Part model, mm, in its own coordinate system. Round coordinates to 2 decimals unless told otherwise and drop trailing zeros. Loops run counter-clockwise (first coordinate to the right, second up) from the corner with the lowest first, then second, coordinate; pieces in that order, holes last. Notation, with made-up numbers: (-17.75, -10) - (35.25, -10) arc R22 ccw to (35.25, 20) - close; hole circle Ø1 at (58.25, 21). An arc over 180 degrees is marked (long way). Write each question's results on one line, items separated by ' | '. Start each with the question number.
(1) Flat gauge pins, fed straight in: P1, Ø6, axis at y = -9, z = -19, coming from the +X side; P2, Ø8, axis at x = 182.5, y = 3, coming from the -Z side; P3, Ø14, axis at x = 18.5, y = 0, coming from the -Z side. Where does each tip first touch, or does it go through?
(2) Drill centre lines: L1, parallel to Y at x = 18, z = -3; L2, parallel to X at y = 0, z = 9; L3, parallel to Y at x = 798, z = -4. Where is each one in solid material? Low to high.
(3) Cut at A-A, the plane x = 598. List the corners of the cut face in (y, z), then the cut area to 3 significant figures.
from build123d import *

# Parameters (mm, degrees)
CHAMFER1_SIZE          = 3.5
CHAMFER2_SIZE          = 1
SKETCH2_R              = 6
CUT_EXTRUDE1_DEPTH     = 50
M12_TAPPED_HOLE1_D     = 10.2
M12_TAPPED_HOLE1_DEPTH = 23.25
M12_TAPPED_HOLE1_TIP   = 3.064389157


with BuildPart() as part:
    # Sketch1 → Revolve1 (revolve)
    with BuildSketch(Plane.XY, mode=Mode.PRIVATE) as revolve1_sk:
        Polygon((81, 19.5), (78, 19.5), (72.5, 25), (38, 25), (38, 22.5), (38, 20.3), (33.5, 20.3), (33.5, 22.5), (0, 22.5), (0, 0), (38, 0), (78, 0), (81, 0), (1010, 0), (1010, 20), (81, 20), align=None)
    revolve(revolve1_sk.sketch.rotate(Axis((38, 0, 0), (1, 0, 0)), 90), axis=Axis((38, 0, 0), (1, 0, 0)))

    # Chamfer1
    chamfer1_edges = [part.edges().sort_by_distance(p)[0] for p in [
        (1010, 0, -20),
    ]]
    chamfer(chamfer1_edges, length=CHAMFER1_SIZE)

    # Chamfer2
    chamfer2_edges = [part.edges().sort_by_distance(p)[0] for p in [
        (0, 0, -22.5),
    ]]
    chamfer(chamfer2_edges, length=CHAMFER2_SIZE)

    # Sketch2 → Cut-Extrude1 (cut, symmetric)
    with BuildSketch(Plane.XY):
        with Locations((18.5, 0)):
            Circle(SKETCH2_R)
    extrude(amount=CUT_EXTRUDE1_DEPTH, both=True, mode=Mode.SUBTRACT)

    # M12 Tapped Hole1
    with Locations(Plane(origin=(1010, 0, 0), x_dir=(0, 0, -1), z_dir=(1, 0, 0))):
        with Locations((0, 0)):
            Hole(M12_TAPPED_HOLE1_D / 2, depth=M12_TAPPED_HOLE1_DEPTH)
            with Locations((0, 0, -(M12_TAPPED_HOLE1_DEPTH + M12_TAPPED_HOLE1_TIP / 2))):  # 118° drill point
                Cone(0, M12_TAPPED_HOLE1_D / 2, M12_TAPPED_HOLE1_TIP, mode=Mode.SUBTRACT)


solid = part.part
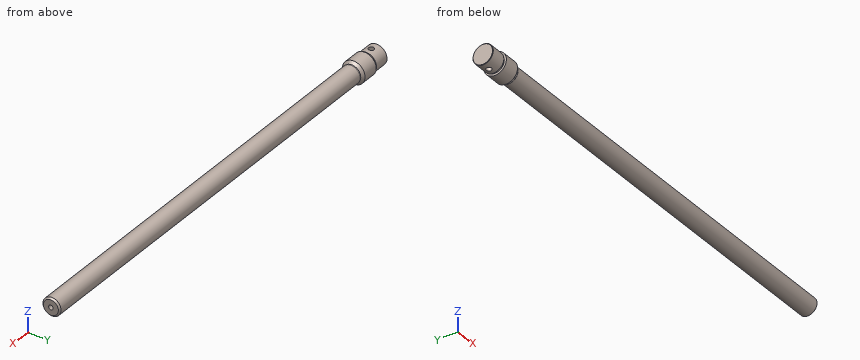
A:
1) P1: x = 1008.48 | P2: z = -20 | P3: z = -22.5
2) L1: -22.3 to -5.98, 5.98 to 22.3 | L2: 0 to 12.5, 24.5 to 1010 | L3: -19.6 to 19.6
3) outline: circle Ø40 at (0, 0) | area: 1,260 mm2
